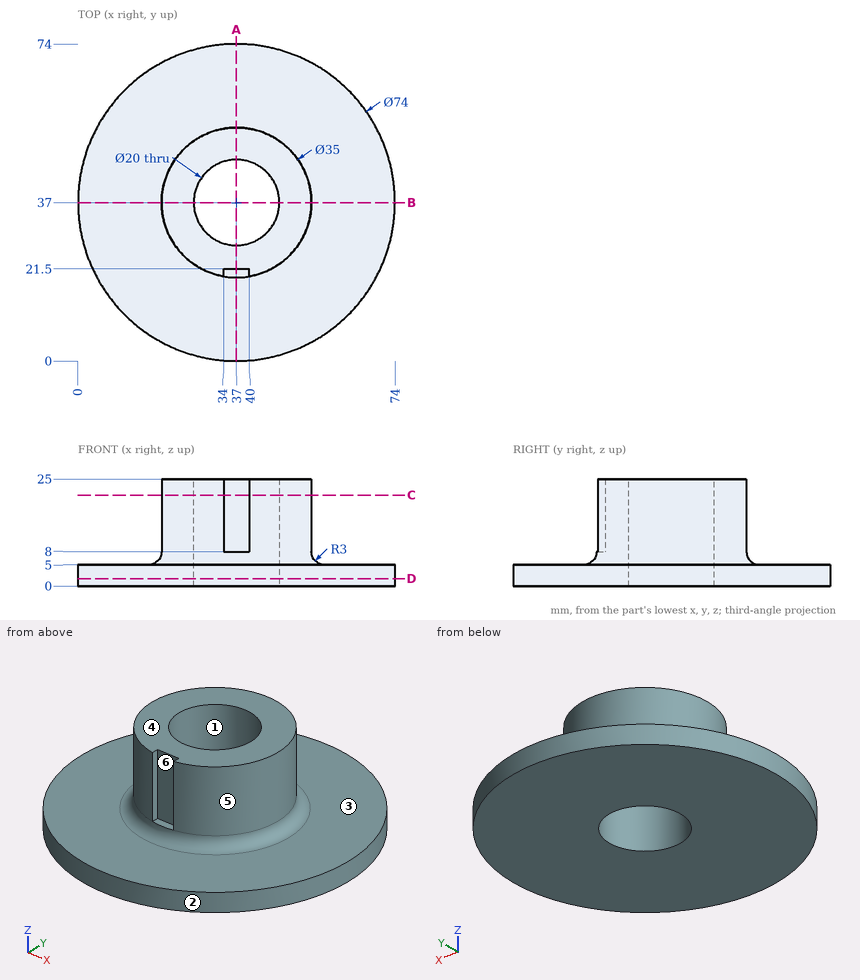
Geometry: see drawing. Coordinates: mm, zero at the bounding-box minimum. A direction names the side the tool comes from. Coordinates: 2 decimals unless noted, no trailing zeros. Order: outer loops, then holes, each group sorted by start corner. A loop starts at its lowest first (then second) coordinate and runs counter-clockwise, first axis right, second up. Notation, with made-up numbers: M 86.25,1 L 111.25,1 A32 cw 111.25,38 Z; hole C -25,71.5 d2. An arc over 180 degrees is marked long. Answer as CSV lines item,"result".
1. Section A-A (x = 37). Return the cut outline in (y, z).
Reported:
outline,"M 0,0 L 27,0 L 27,25 L 21.5,25 L 21.5,8 L 19.5,8 A3 cw 16.5,5 L 0,5 Z; M 47,0 L 74,0 L 74,5 L 57.5,5 A3 cw 54.5,8 L 54.5,25 L 47,25 Z"
2. Access query for the marked faces 4, 5 and 6. Directions: +Z, -Z, +X, -X, +Y, -Y. A direction counts if a zero-diameter tool reaches every point of the face in a straight line with its end or side. Return the directions, or none.
Reported:
face 4,"+Z, +X, -X, +Y, -Y"
face 5,"+Z"
face 6,"+Z, -Y"
3. First-contact query: P1, Ø4, axis at y = 51, z = 15.5, coming from the +X side; P2, Ø10, axis at x = 47.5, z = 6, coming from the +Y side; P3, Ø3, axis at x = 37, z = 18, coming from the -Y side; P4, Ø2, axis at x = 37.5, y = 21, coming from the +Z side. Flat tips, straight axial feed; report the tip coordinate or a pass-through.
Reported:
P1,"x = 49.74"
P2,"y = 73.57"
P3,"y = 21.5"
P4,"z = 25"
4. Section C-C (z = 21.25). Return the cut outline in (x, y).
Reported:
outline,"M 34,19.76 L 34,21.5 L 40,21.5 L 40,19.76 A17.5 ccw long Z; hole C 37,37 d20"
5. Pull-direction query (X, two-part tool) for the marked faces 1, 2 and 3; classes: released by +X, released by -X, zero draft, split by the parting line, or undercut.
Reported:
face 1,"undercut"
face 2,"split by the parting line"
face 3,"zero draft"
6. Section D-D (z = 1.75). Return the cut outline in (x, y).
Reported:
outline,"C 37,37 d74; hole C 37,37 d20"
7. Material intervals for line 1 (Y direction, x = 37, z = 9); line 2 (X direction, y = 41, z = 22.75); line 3 (Y direction, x = 28, z = 8.75), sorted ascending. Write a range as from..to.
Reported:
line 1,"21.5..27, 47..54.5"
line 2,"19.96..27.83, 46.17..54.04"
line 3,"21.99..32.64, 41.36..52.01"
8. Section B-B (y = 37). Return the cut outline in (x, z), then the cut area to 3 significant figures.
Reported:
outline,"M 0,0 L 27,0 L 27,25 L 19.5,25 L 19.5,8 A3 cw 16.5,5 L 0,5 Z; M 47,0 L 74,0 L 74,5 L 57.5,5 A3 cw 54.5,8 L 54.5,25 L 47,25 Z"
area,"574 mm2"
